The listing builds one solid part. Answer for the finished solid, in the listing's coordinates (mm). A direction names the side the tool comes from. Give positions to 0.01 mm unless a question says otherwise; leave off trailing zeros. Order: outer loops, then holes, each group sorted by start corner. A loop starts at its lowest first (then second) coordinate and runs counter-clockwise, first axis right, second up. Notation, with made-up numbers: (51.25, 15) - (61.25, 15) arc R24 ccw to (61.25, 39) - close; hole circle Ø9 at (46.5, 12.5). An arc over 180 degrees is marked (long way). Use CSV: the item, a comma, the result in double quotes.
```python
from build123d import *

# Parameters (mm, degrees)
FILLET3_R = 0.1


with BuildPart() as part:
    # Sketch1 → Revolve1 (revolve)
    with BuildSketch(Plane.XY, mode=Mode.PRIVATE) as revolve1_sk:
        Polygon((-3.5, 0), (-2.02328752, 0), (-2.02328752, -11.6), (-1, -11.6), (-1, 10.4), (-3, 10.4), (-3, 1), (-3.5, 1), align=None)
    revolve(revolve1_sk.sketch.rotate(Axis((0, -19.747048695, 0), (0, 1, 0)), 270), axis=Axis((0, -19.747048695, 0), (0, 1, 0)))

    # Fillet3
    fillet3_edges = [part.edges().sort_by_distance(p)[0] for p in [
        (0, 10.4, 3),
    ]]
    fillet(fillet3_edges, radius=FILLET3_R)


solid = part.part
```
Item 1: Find the intervals of material crossed by line 1 along X through (y, z) = (-3, 0); line 2 along X through (y, z) = (4.5, 0); line 3 along Y through (x, z) = (-3, 1.5), in increasing order.
Taken from the geometry:
line 1,"-2.02 to -1, 1 to 2.02"
line 2,"-3 to -1, 1 to 3"
line 3,"0 to 1"
Item 2: The part is cut by section A-A (x = 0). Give the vertices of the cut face in (y, z).
Taken from the geometry:
outline,"(-11.6, -2.02) - (0, -2.02) - (0, -3.5) - (1, -3.5) - (1, -3) - (10.3, -3) arc R0.1 ccw to (10.4, -2.9) - (10.4, -1) - (-11.6, -1) - close; (-11.6, 1) - (10.4, 1) - (10.4, 2.9) arc R0.1 ccw to (10.3, 3) - (1, 3) - (1, 3.5) - (0, 3.5) - (0, 2.02) - (-11.6, 2.02) - close"
Item 3: The part is cut by section B-B (z = 0). Give the vertices of the cut face in (x, y), and give its area (3 significant figures).
Taken from the geometry:
outline,"(-3.5, 0) - (-2.02, 0) - (-2.02, -11.6) - (-1, -11.6) - (-1, 10.4) - (-2.9, 10.4) arc R0.1 ccw to (-3, 10.3) - (-3, 1) - (-3.5, 1) - close; (1, -11.6) - (2.02, -11.6) - (2.02, 0) - (3.5, 0) - (3.5, 1) - (3, 1) - (3, 10.3) arc R0.1 ccw to (2.9, 10.4) - (1, 10.4) - close"
area,"66.3 mm^2"
Item 4: Each of these flat-tipped pins is pushed along its axis until it touches: pin 1 (2 mm diameter, centred on x = 0.5, y = -1.5, fed in from +Z); pin 2 (1.5 mm diameter, centred on y = -4.5, z = 1, fed in from -X); pin 3 (1.5 mm diameter, centred on y = -2.5, z = 1.5, fed in from +X). Where does it stop, or does it pass through?
Taken from the geometry:
pin 1,"z = 2.02"
pin 2,"x = -2.01"
pin 3,"x = 1.88"
Item 5: Which of the six approach directions +Z, -Z, +X, -X, +Y, -Y give full straight-line access (tool end or side, diameter ignored) to faces 4 (the face through (3.417, 0.493, 0.759)), 5 (the face through (2, 0, -2)), 6 (the face through (-1, 1, 3))?
Taken from the geometry:
face 4,"+Y, -Y"
face 5,"-Y"
face 6,"+Y"
Item 6: The part is cut by section C-C (y = 5). Give the vertices of the cut face in (x, z), and give its area (3 significant figures).
Taken from the geometry:
outline,"circle Ø6 at (0, 0); hole circle Ø2 at (0, 0)"
area,"25.1 mm^2"
Item 7: The part is cut by section D-D (y = -3.75). Give the vertices of the cut face in (x, z).
Taken from the geometry:
outline,"circle Ø4.05 at (0, 0); hole circle Ø2 at (0, 0)"
Item 8: The mould has two halves that part along Z. Classify faces 1 (the face through (1, 0, 0)), 2 (the face through (1, -11.6, -1)), 3 (the face through (1.231, -5.881, 1.606)): +Z half, -Z half, draft (parallel to the pull), parting line (faces both ways), or undercut.
Taken from the geometry:
face 1,"undercut"
face 2,"draft"
face 3,"parting line"
